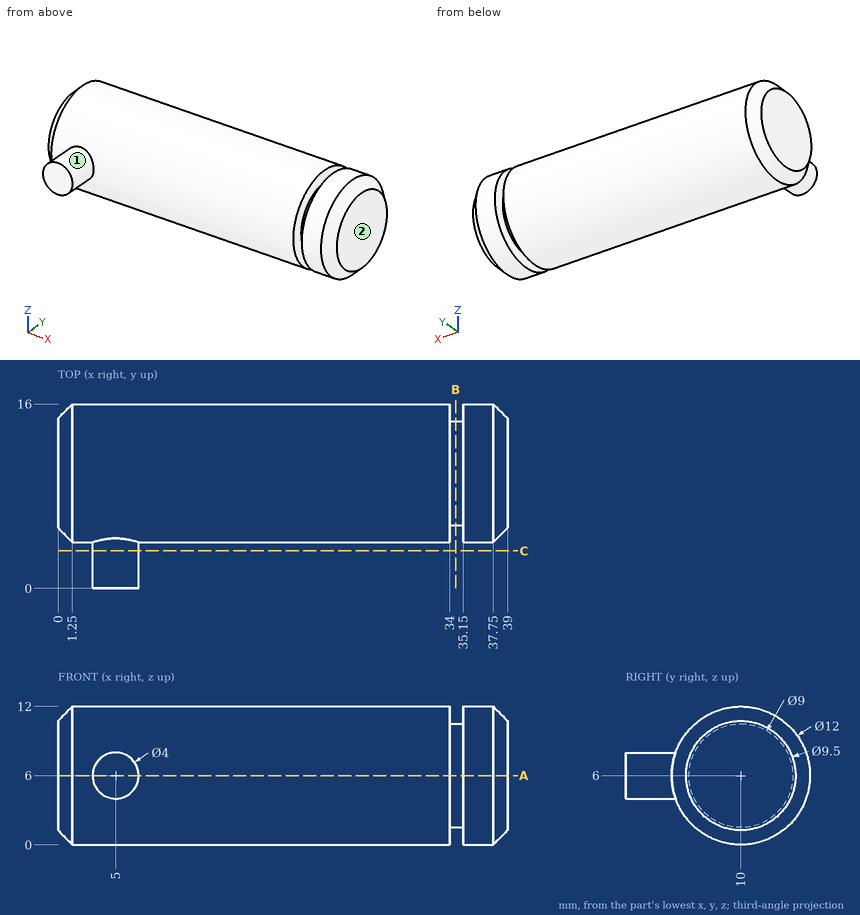
For this review, use the dimensioned drawing (mm, ordinates from the lowest corner) and the shaded views. A direction names the side the tool comes from. Round coordinates to 2 decimals unless told otherwise and drop trailing zeros. Write each loop counter-clockwise with the first axis right and the second up, starting at its lowest first coordinate (ties: lowest second). Pieces come first, ordered by that corner, then holes. Notation, with made-up numbers: (55, 16.25) -> (76, 16.25) arc R16 ccw to (76, 24.25) -> close; hole circle Ø6 at (-18, 21). An arc over 180 degrees is marked (long way). One line per item, written item: value. Start each with the question number.
Q1. Insertion check: P1, Ø6, axis at x = 29, z = 10, coming from the +Y side; P2, Ø3, axis at x = 34.5, z = 4.5, coming from the -Y side. Each pin has a flat end and moves straight along its axis. Give the tip position at first contact, or say it passes through.
Q2. Add section C-C (y = 3.25). Give the boundary of the cut face in (x, z), then the cut area to 3 significant figures.
Q3. Add section B-B (x = 34.5). Give the boundary of the cut face in (y, z), then the cut area to 3 significant figures.
Q4. Add section A-A (z = 6). Give the boundary of the cut face in (x, y).
Q5. Tool access review of the marked faces 1 and 2: name each direction out of +Z, -Z, +X, -X, +Y, -Y from which nothing blocks a thin tool from reaching the whole face with its end or side.
Q6. To check wall thickness, follow probe 1 along X at (y, z) = (8.5, 1); probe 2 along Y at (x, z) = (11.5, 11.25); probe 3 along X at (y, z) = (15, 8.5). State the ranges of each line that lie inside material, in increasing order.
Response:
1. P1: stops at y = 15.92
1. P2: stops at y = 4
2. outline: circle Ø4 at (5, 6)
2. area: 12.6 mm^2
3. outline: circle Ø9 at (10, 6)
3. area: 63.6 mm^2
4. outline: (0, 5.25) -> (1.25, 4) -> (3, 4) -> (3, 0) -> (7, 0) -> (7, 4) -> (34, 4) -> (34, 5.5) -> (35.15, 5.5) -> (35.15, 4) -> (37.75, 4) -> (39, 5.25) -> (39, 14.75) -> (37.75, 16) -> (35.15, 16) -> (35.15, 14.5) -> (34, 14.5) -> (34, 16) -> (1.25, 16) -> (0, 14.75) -> close
5. face 1: -Y
5. face 2: +Z, -Z, +X, +Y, -Y
6. probe 1: x = 0.47 to 34, 35.15 to 38.53
6. probe 2: y = 7.1 to 12.9
6. probe 3: x = 0.84 to 34, 35.15 to 38.16
